from build123d import *

# Parameters (mm, degrees)
BOSS_EXTRUDE1_DEPTH                                = 48
SKETCH2_R                                          = 15
CUT_EXTRUDE1_DEPTH                                 = 93.349417704
HOLE_SIZE_PER_HEX_SOCKET_CAP_SCREW_TYP_D           = 5.5
HOLE_SIZE_PER_HEX_SOCKET_CAP_SCREW_TYP_CBORE_D     = 10
HOLE_SIZE_PER_HEX_SOCKET_CAP_SCREW_TYP_CBORE_DEPTH = 5.7
CHAMFER1_SIZE                                      = 3
SKETCH6_R                                          = 2.8
CUT_EXTRUDE2_DEPTH                                 = 48


with BuildPart() as part:
    # Sketch1 → Boss-Extrude1 (new body)
    with BuildSketch(Plane.XY):
        Polygon((-9.247374932, 66.146919431), (-9.247374932, -21.853080569), (-52.247374932, -21.853080569), (-52.247374932, -33.853080569), (5.752625068, -33.853080569), (5.752625068, 66.146919431), align=None)
    extrude(amount=BOSS_EXTRUDE1_DEPTH)

    # Sketch2 → Cut-Extrude1 (cut, through all)
    with BuildSketch(Plane.ZY.offset(9.247374932)):
        with Locations((24, 38.146919431)):
            Circle(SKETCH2_R)
    extrude(amount=-CUT_EXTRUDE1_DEPTH, mode=Mode.SUBTRACT)

    # Hole size (per) hex socket cap screw type 1 (through all)
    with Locations(Plane.ZY.offset(9.247374932)):
        with Locations((7, 55.146919431), (41, 55.146919431), (41, 21.146919431), (7, 21.146919431)):
            CounterBoreHole(HOLE_SIZE_PER_HEX_SOCKET_CAP_SCREW_TYP_D / 2, HOLE_SIZE_PER_HEX_SOCKET_CAP_SCREW_TYP_CBORE_D / 2, HOLE_SIZE_PER_HEX_SOCKET_CAP_SCREW_TYP_CBORE_DEPTH)

    # Chamfer1
    chamfer1_edges = [part.edges().sort_by_distance(p)[0] for p in [
        (-52.247374932, -27.853080569, 48),
        (-1.747374932, 66.146919431, 48),
        (-52.247374932, -27.853080569, 0),
        (-1.747374932, 66.146919431, 0),
    ]]
    chamfer(chamfer1_edges, length=CHAMFER1_SIZE)

    # Sketch6 → Cut-Extrude2 (cut)
    with BuildSketch(Plane(origin=(0, -21.853080569, 0), x_dir=(1, 0, 0), z_dir=(0, 1, 0))):
        with Locations(Location((-42.810470963, -9, 0), (0, 0, 180))):
            Circle(SKETCH6_R)
        with Locations(Location((-22.810470963, -9, 0), (0, 0, 180))):
            Circle(SKETCH6_R)
        with Locations(Location((-42.810470963, -39, 0), (0, 0, 180))):
            Circle(SKETCH6_R)
        with Locations(Location((-22.810470963, -39, 0), (0, 0, 180))):
            Circle(SKETCH6_R)
    extrude(amount=-CUT_EXTRUDE2_DEPTH, mode=Mode.SUBTRACT)


solid = part.part
Design review of the part built by this model. Coordinates are the model's own, in mm. A direction names the side the tool comes from. Coordinates: 2 decimals unless noted, no trailing zeros. Loops run counter-clockwise (first coordinate to the right, second up) from the corner with the lowest first, then second, coordinate; pieces in that order, holes last. Notation, with made-up numbers: (64.5, 8) -> (92.5, 8) arc R22 ccw to (92.5, 29) -> close; hole circle Ø6 at (32, 63). An arc over 180 degrees is marked (long way). Use a Markdown table: item, result. Add a question column.
Item 1: Wall thickness on L1, parallel to Y at x = -3.25, z = 24; L2, parallel to Z at x = -5, y = 51; L3, parallel to X at y = 17.5, z = 18.5: over which ranges is each line inside the solid? List them lowest first. Write a range as from..to.
Item 2: We need section D-D, the plane y = -23.5. Write out the cut boundary in (x, z), and give its area (3 significant figures).
Item 3: Clearance check with flat-ended pins moving along their axes: P1, Ø2, axis at y = 24, z = 15, coming from the -X side; P2, Ø6.5, axis at y = 21.15, z = 7, coming from the -X side; P3, Ø9, axis at x = -22.81, z = 39, coming from the +Y side. State where each tip first meets the part, or that it passes through.
Item 4: We need section B-B, the plane y = 28. Write out the cut boundary in (x, z).
Item 5: The part is to be moulded in two halves that separate along X. For faces 4 (the flat face through (-1.642, 64.626, 46.521)), 5 (the flat face through (5.753, 15, 24)), 6 (the cylindrical face through (-44.103, -27.769, 36.516)), say which applies: +X half, -X half, draft (parallel to the pull), parting line (faces both ways), or undercut.
Item 6: Machinability: for faces 1 (the flat face through (-3.547, 19, 9)), 2 (the flat face through (-30, -21.853, 24)), 3 (the cylindrical face through (-45.4, -27.77, 7.93)), which of the approach directions +Z, -Z, +X, -X, +Y, -Y give a long, thin tool a straight path to every point of the face, cutting with its end or side? Answer none if there is none.
Item 7: We need section A-A, the plane z = 24. Write out the cut boundary in (x, y), and give its area (3 significant figures).
Item 8: We need section C-C, the plane z = 7.5. Count the separate pieces of the cut face and the enclosed holes in it, and give its area (3 significant figures).
Numbers:
| question | item | result |
|---|---|---|
| 1 | L1 | y = -33.85..23.15, 53.15..66.15 |
| 1 | L2 | z = 0..4.21, 9.79..16.27, 31.73..38.21, 43.79..48 |
| 1 | L3 | x = -9.25..5.75 |
| 2 | outline | (-52.25, 3) -> (-49.25, 0) -> (5.75, 0) -> (5.75, 48) -> (-49.25, 48) -> (-52.25, 45) -> close; hole circle Ø5.6 at (-42.81, 9); hole circle Ø5.6 at (-42.81, 39); hole circle Ø5.6 at (-22.81, 9); hole circle Ø5.6 at (-22.81, 39) |
| 2 | area | 2,680 mm^2 |
| 3 | P1 | stops at x = -9.25 |
| 3 | P2 | stops at x = -3.55 |
| 3 | P3 | stops at y = -21.85 |
| 4 | outline | (-9.25, 0) -> (5.75, 0) -> (5.75, 12.95) -> (-9.25, 12.95) -> close; (-9.25, 35.05) -> (5.75, 35.05) -> (5.75, 48) -> (-9.25, 48) -> close |
| 5 | face 4 | draft |
| 5 | face 5 | +X half |
| 5 | face 6 | undercut |
| 6 | face 1 | -X |
| 6 | face 2 | +Z, -Z, -X, +Y |
| 6 | face 3 | +Y, -Y |
| 7 | outline | (-52.25, -33.85) -> (5.75, -33.85) -> (5.75, 23.15) -> (-9.25, 23.15) -> (-9.25, -21.85) -> (-52.25, -21.85) -> close; (-9.25, 53.15) -> (5.75, 53.15) -> (5.75, 66.15) -> (-9.25, 66.15) -> close |
| 7 | area | 1,570 mm^2 |
| 8 | separate pieces | 5 |
| 8 | enclosed holes | 0 |
| 8 | area | 1,690 mm^2 |
